Geometry check sheet. Reference: the model listing, model coordinates, mm. A direction names the side the tool comes from. Round coordinates to 2 decimals unless told otherwise and drop trailing zeros. Order: outer loops, then holes, each group sorted by start corner. A loop starts at its lowest first (then second) coordinate and runs counter-clockwise, first axis right, second up. Notation, with made-up numbers: M -33.5,65.25 L 13.5,65.25 A28 cw 13.5,87.25 Z; hole C -7,24 d10. An arc over 180 degrees is marked long. Return JSON: item names as keys, results as strings. Group by question number.
```python
from build123d import *

# Parameters (mm, degrees)
SKETCH1_W                                           = 66
SKETCH1_H                                           = 160
BOSS_EXTRUDE1_DEPTH                                 = 15
CBORE_FOR_M6_HEX_SOCKET_HEAD_CAP_SCREW1_D           = 6.6
CBORE_FOR_M6_HEX_SOCKET_HEAD_CAP_SCREW1_CBORE_D     = 11
CBORE_FOR_M6_HEX_SOCKET_HEAD_CAP_SCREW1_CBORE_DEPTH = 6.4
MOVE_FACE1_BY                                       = 110
M5_TAPPED_HOLE1_D                                   = 4.2
SKETCH6_R                                           = 3.5
CUT_EXTRUDE1_DEPTH                                  = 1.6
CHAMFER2_SIZE                                       = 1
CHAMFER1_SIZE                                       = 3
SKETCH12_R                                          = 3
CUT_EXTRUDE2_DEPTH                                  = 279.354091042


with BuildPart() as part:
    # Sketch1 → Boss-Extrude1 (new body)
    with BuildSketch(Plane.XY):
        with Locations((33, 80)):
            Rectangle(SKETCH1_W, SKETCH1_H)
    extrude(amount=BOSS_EXTRUDE1_DEPTH)

    # CBORE for M6 Hex Socket Head Cap Screw1 (through all)
    with Locations(Plane(origin=(0, 0, 0), x_dir=(-1, 0, 0), z_dir=(0, 0, -1))):
        with Locations((-53, 15), (-13, 15), (-53, 145), (-13, 145)):
            CounterBoreHole(CBORE_FOR_M6_HEX_SOCKET_HEAD_CAP_SCREW1_D / 2, CBORE_FOR_M6_HEX_SOCKET_HEAD_CAP_SCREW1_CBORE_D / 2, CBORE_FOR_M6_HEX_SOCKET_HEAD_CAP_SCREW1_CBORE_DEPTH)

    # Move Face1: a face moved outward by 110.0
    extrude(part.faces().sort_by_distance((33, 160, 7.5))[0], amount=MOVE_FACE1_BY, dir=(0, 1, 0))

    # M5 Tapped Hole1 (through all)
    with Locations(Plane(origin=(0, 0, 0), x_dir=(-1, 0, 0), z_dir=(0, 0, -1))):
        with Locations((-39.3, 244.5), (-39.3, 174.5), (-39.3, 224.5), (-39.3, 194.5)):
            Hole(M5_TAPPED_HOLE1_D / 2)

    # Sketch6 → Cut-Extrude1 (cut)
    with BuildSketch(Plane(origin=(0, 0, 0), x_dir=(-1, 0, 0), z_dir=(0, 0, -1))):
        with Locations((-39.3, 244.5)):
            Circle(SKETCH6_R)
        with Locations((-39.3, 174.5)):
            Circle(SKETCH6_R)
    extrude(amount=-CUT_EXTRUDE1_DEPTH, mode=Mode.SUBTRACT)

    # Chamfer2
    chamfer2_edges = [part.edges().sort_by_distance(p)[0] for p in [
        (66, 135, 15),
        (0, 135, 15),
        (66, 135, 0),
        (0, 135, 0),
    ]]
    chamfer(chamfer2_edges, length=CHAMFER2_SIZE)

    # Chamfer1
    chamfer1_edges = [part.edges().sort_by_distance(p)[0] for p in [
        (0, 0, 7.5),
        (66, 0, 7.5),
        (0, 270, 7.5),
        (66, 270, 7.5),
    ]]
    chamfer(chamfer1_edges, length=CHAMFER1_SIZE)

    # Sketch12 → Cut-Extrude2 (cut, through all)
    with BuildSketch(Plane(origin=(0, 0, 0), x_dir=(-1, 0, 0), z_dir=(0, 0, -1))):
        with Locations((-33, 145)):
            Circle(SKETCH12_R)
        with Locations((-33, 15)):
            Circle(SKETCH12_R)
    extrude(amount=-CUT_EXTRUDE2_DEPTH, mode=Mode.SUBTRACT)


solid = part.part
```
Q1. Section check A-A on x = 13. Record the cut outline in (y, z).
Q2. Set-up check for faces 1 (the face through (12.28, 141.78, 10.76)), 2 (the face through (57.05, 148.72, 3.16)): record each of +Z, -Z, +X, -X, +Y, -Y from which the full face is reachable in a straight line by a thin tool's end or side.
Q3. Section check C-C on x = 33. Record the cut outline in (y, z), plus the area to 3 significant figures.
Q4. Section check B-B on y = 145. Record the cut outline in (x, z), plus the area to 3 significant figures.
Q5. Depth check by flat-ended pin: pin 1 Ø3.5 at (x, y) = (12, 12.5) entering from -Z; pin 2 Ø5 at (x, y) = (33, 145) entering from -Z; pin 3 Ø5.5 at (x, y) = (39.3, 174.5) entering from -Z. Enter the tip coordinate at first touch or a pass-through.
Q6. Release check for a two-part mould opening along X. For faces 3 (the face through (33, 133, 15)), 4 (the face through (39.027, 246.582, 8.394)), 5 (the face through (66, 133, 7)) record: +X half, -X half, draft (parallel to the pull), parting line (faces both ways), or undercut.
Q7. Material ranges on line 1 along Y through (x, z) = (53, 12.5); line 2 along Y through (x, z) = (53, 3); line 3 along Y through (x, z) = (39.3, 1.15), recorded low to high.
Geometry check:
{
 "1": {"outline": "M 0,0 L 9.5,0 L 9.5,6.4 L 11.7,6.4 L 11.7,15 L 0,15 Z; M 18.3,6.4 L 20.5,6.4 L 20.5,0 L 139.5,0 L 139.5,6.4 L 141.7,6.4 L 141.7,15 L 18.3,15 Z; M 148.3,6.4 L 150.5,6.4 L 150.5,0 L 270,0 L 270,15 L 148.3,15 Z"},
 "2": {"face 1": "+Z, -Z", "face 2": "-Z"},
 "3": {"outline": "M 0,0 L 12,0 L 12,15 L 0,15 Z; M 18,0 L 142,0 L 142,15 L 18,15 Z; M 148,0 L 270,0 L 270,15 L 148,15 Z", "area": "3,870 mm^2"},
 "4": {"outline": "M 0,1 L 1,0 L 7.5,0 L 7.5,6.4 L 9.7,6.4 L 9.7,15 L 1,15 L 0,14 Z; M 16.3,6.4 L 18.5,6.4 L 18.5,0 L 30,0 L 30,15 L 16.3,15 Z; M 36,0 L 47.5,0 L 47.5,6.4 L 49.7,6.4 L 49.7,15 L 36,15 Z; M 56.3,6.4 L 58.5,6.4 L 58.5,0 L 65,0 L 66,1 L 66,14 L 65,15 L 56.3,15 Z", "area": "644 mm^2"},
 "5": {"pin 1": "stops at z = 6.4", "pin 2": "passes through", "pin 3": "stops at z = 1.6"},
 "6": {"face 3": "draft", "face 4": "undercut", "face 5": "+X half"},
 "7": {"line 1": "y = 0 to 11.7, 18.3 to 141.7, 148.3 to 270", "line 2": "y = 0 to 9.5, 20.5 to 139.5, 150.5 to 270", "line 3": "y = 0 to 171, 178 to 192.4, 196.6 to 222.4, 226.6 to 241, 248 to 270"}
}
